Source: CAD feature listing. Evaluate the final solid. Frame: model axes, mm. A direction names the side the tool comes from. Give positions to 0.01 mm unless a question says otherwise; leave off trailing zeros. Loops run counter-clockwise (first coordinate to the right, second up) from the corner with the lowest first, then second, coordinate; pieces in that order, holes last. Notation, with made-up numbers: M 85,70 L 118,70 A24 ccw 118,90 Z; hole C 87.5,15 d4. An arc over 180 degrees is marked long. Write item = value, one per line.
from build123d import *

# Parameters (mm, degrees)
SKETCH_1_W              = 80
SKETCH_1_H              = 150
SKETCH_1_R              = 20
EXTRUDE_1_DEPTH         = 35
CHAMFER_1_SIZE          = 0.5
HOLE_WIZARD_M12_1_D     = 10.2
HOLE_WIZARD_M12_1_DEPTH = 29.25
HOLE_WIZARD_M12_1_TIP   = 3.064389157
HOLE_WIZARD_M12_2_D     = 10.2
HOLE_WIZARD_M12_2_DEPTH = 29.25
HOLE_WIZARD_M12_2_TIP   = 3.064389157


with BuildPart() as part:
    # 草图1 → 凸台-拉伸1 (new body)
    with BuildSketch(Plane(origin=(0, 0, 0), x_dir=(1, 0, 0), z_dir=(0, 1, 0))):
        Rectangle(SKETCH_1_W, SKETCH_1_H)
        with Locations(Location((0, 0, 0), (0, 0, 270))):
            Circle(SKETCH_1_R, mode=Mode.SUBTRACT)
    extrude(amount=EXTRUDE_1_DEPTH)

    # 倒角1
    chamfer_1_edges = [part.edges().sort_by_distance(p)[0] for p in [
        (-40, 35, 0),
        (0, 0, -20),
        (0, 35, -20),
        (0, 35, 75),
        (40, 35, 0),
        (0, 0, 75),
        (-40, 0, 0),
        (0, 0, -75),
        (40, 0, 0),
        (0, 35, -75),
        (40, 17.5, 75),
        (-40, 17.5, 75),
        (-40, 17.5, -75),
        (40, 17.5, -75),
    ]]
    chamfer(chamfer_1_edges, length=CHAMFER_1_SIZE)

    # M12 螺纹孔1
    with Locations(Plane.XY.offset(75)):
        with Locations((25, 17.5), (-25, 17.5)):
            Hole(HOLE_WIZARD_M12_1_D / 2, depth=HOLE_WIZARD_M12_1_DEPTH)
            with Locations((0, 0, -(HOLE_WIZARD_M12_1_DEPTH + HOLE_WIZARD_M12_1_TIP / 2))):  # 118° drill point
                Cone(0, HOLE_WIZARD_M12_1_D / 2, HOLE_WIZARD_M12_1_TIP, mode=Mode.SUBTRACT)

    # M12 螺纹孔2
    with Locations(Plane(origin=(0, 0, -75), x_dir=(-1, 0, 0), z_dir=(0, 0, -1))):
        with Locations((-25, 17.5), (25, 17.5)):
            Hole(HOLE_WIZARD_M12_2_D / 2, depth=HOLE_WIZARD_M12_2_DEPTH)
            with Locations((0, 0, -(HOLE_WIZARD_M12_2_DEPTH + HOLE_WIZARD_M12_2_TIP / 2))):  # 118° drill point
                Cone(0, HOLE_WIZARD_M12_2_D / 2, HOLE_WIZARD_M12_2_TIP, mode=Mode.SUBTRACT)


solid = part.part
1. Cut plane D-D, the plane z = -63. Return the cut outline in (x, y).
Derived:
outline = M -40,0.5 L -39.5,0 L 39.5,0 L 40,0.5 L 40,34.5 L 39.5,35 L -39.5,35 L -40,34.5 Z; hole C -25,17.5 d10.2; hole C 25,17.5 d10.2
2. First-contact query: pin 1 Ø8 at (x, y) = (-25, 17.5) entering from +Z; pin 2 Ø6 at (x, y) = (25, 17.5) entering from +Z. Flat tips, straight axial feed; report the tip coordinate or a pass-through.
Derived:
pin_1 = 45.09
pin_2 = 44.49
3. Cut plane B-B, the plane x = 0. Return the cut outline in (y, z), then the cut area to 3 significant figures.
Derived:
outline = M 0,-74.5 L 0.5,-75 L 34.5,-75 L 35,-74.5 L 35,-20.5 L 34.5,-20 L 0.5,-20 L 0,-20.5 Z; M 0,20.5 L 0.5,20 L 34.5,20 L 35,20.5 L 35,74.5 L 34.5,75 L 0.5,75 L 0,74.5 Z
area = 3,850 mm²
4. Reachability of faces 5 (the flat face through (-1, 17, 75)), 6 (the cylindrical face through (20.95, 14.4, -60.17)), 7 (the cylindrical face through (29.05, 14.4, 60.17)) from +Z, -Z, +X, -X, +Y, -Y: full face, straight path, thin tool, end or side. Return the list, or none.
Derived:
face_5 = +Z, +X, -X, +Y, -Y
face_6 = -Z
face_7 = +Z
5. Cut plane C-C, the plane y = 3. Return the cut outline in (x, z), then the cut area to 3 significant figures.
Derived:
outline = M -40,-74.5 L -39.5,-75 L 39.5,-75 L 40,-74.5 L 40,74.5 L 39.5,75 L -39.5,75 L -40,74.5 Z; hole C 0,0 d40
area = 10,700 mm²
6. Pull-direction query (Y, two-part tool) for faces 1 (the flat face through (17, 0, -18)), 2 (the flat face through (17, 35, -18)), 3 (the conical face through (24.2, 17.8, -43.2)), 4 (the flat face through (40, 17, 1)); classes: +Y half, -Y half, draft (parallel to the pull), parting line (faces both ways), or undercut.
Derived:
face_1 = -Y half
face_2 = +Y half
face_3 = undercut
face_4 = draft
7. Material intervals for probe 1 along X at (y, z) = (17, -52); probe 2 along Y at (x, z) = (25, -51.75); probe 3 along X at (y, z) = (15, 0), sorted ascending. Write a range as from..to.
Derived:
probe_1 = -40..-30.08, -19.92..19.92, 30.08..40
probe_2 = 0..12.4, 22.6..35
probe_3 = -40..-20, 20..40
8. Cut plane A-A, the plane z = 0. Return the cut outline in (x, y), then the cut area to 3 significant figures.
Derived:
outline = M -40,0.5 L -39.5,0 L -20.5,0 L -20,0.5 L -20,34.5 L -20.5,35 L -39.5,35 L -40,34.5 Z; M 20,0.5 L 20.5,0 L 39.5,0 L 40,0.5 L 40,34.5 L 39.5,35 L 20.5,35 L 20,34.5 Z
area = 1,400 mm²
